Geometry check sheet. Reference: the model listing, model coordinates, mm. Coordinates: 2 decimals unless noted, no trailing zeros. Loops run counter-clockwise (first coordinate to the right, second up) from the corner with the lowest first, then second, coordinate; pieces in that order, holes last. Notation, with made-up numbers: (43, 40.5) - (52, 40.5) arc R14 cw to (52, 60.5) - close; hole circle Ø4 at (45, -37). An arc over 180 degrees is marked (long way). Write each question's results on one line, items separated by ' | '. Start each with the question number.
(1) Sectioned sample at C-C (y = 0). Enter the section's corners in (x, z), plus the area to 3 significant figures.
(2) Material ranges on probe 1 along Y at (x, z) = (19.6, -22); probe 2 along Y at (x, z) = (19.4, 26); probe 3 along Y at (x, z) = (19.35, 23), recorded low to high.
(3) Sectioned sample at B-B (x = 19.8). Enter the section's corners in (y, z), plus the area to 3 significant figures.
(4) Go/stop test with a flat-tipped pin: pin 1 Ø2.5 at (y, z) = (19, -28) entering from +X. Record where the tip stops, or that it passes through.
(5) Sectioned sample at A-A (z = 24). Enter the section's corners in (x, y).
from build123d import *

# Parameters (mm, degrees)
SKETCH_1_W                = 65
SKETCH_1_H                = 48
EXTRUDE_1_DEPTH           = 20
SKETCH_2_W                = 6
SKETCH_2_H                = 27.1
CUT_EXTRUDE_1_DEPTH       = 80
CUT_EXTRUDE_2_DEPTH       = 80
SKETCH_4_R                = 1.2
CUT_EXTRUDE_3_DEPTH       = 6
HOLE_WIZARD_1_D           = 3.4
HOLE_WIZARD_1_CBORE_D     = 6
HOLE_WIZARD_1_CBORE_DEPTH = 5
FILLET_1_R                = 5
SKETCH_9_W                = 19.082133463
SKETCH_9_H                = 84.157101427
CUT_EXTRUDE_6_DEPTH       = 120
SKETCH_10_W               = 25.015989719
SKETCH_10_H               = 30.267159573
EXTRUDE_2_DEPTH           = 1
SKETCH_11_R               = 1.6
CUT_EXTRUDE_7_DEPTH       = 120
FILLET_2_R                = 2


with BuildPart() as part:
    # 草图1 → 凸台-拉伸1 (new body)
    with BuildSketch(Plane(origin=(0, 0, 0), x_dir=(0, 0, -1), z_dir=(1, 0, 0))):
        Rectangle(SKETCH_1_W, SKETCH_1_H)
    extrude(amount=EXTRUDE_1_DEPTH)

    # 草图2 → 切除-拉伸1 (cut)
    with BuildSketch(Plane(origin=(0, 0, -32.5), x_dir=(-1, 0, 0), z_dir=(0, 0, -1))):
        Rectangle(SKETCH_2_W, SKETCH_2_H)
    extrude(amount=-CUT_EXTRUDE_1_DEPTH, mode=Mode.SUBTRACT)

    # 草图3 → 切除-拉伸2 (cut)
    with BuildSketch(Plane(origin=(20, 0, 0), x_dir=(0, 0, -1), z_dir=(1, 0, 0))):
        Polygon((-26.5, -9), (-21.5, -9), (-21.5, 9), (-26.5, 9), (-26.5, 5.5), (-32.5, 5.5), (-32.5, -5.5), (-26.5, -5.5), align=None)
    extrude(amount=-CUT_EXTRUDE_2_DEPTH, mode=Mode.SUBTRACT)

    # 草图4 → 切除-拉伸3 (cut)
    with BuildSketch(Plane(origin=(20, 0, 0), x_dir=(0, 0, -1), z_dir=(1, 0, 0))):
        with Locations((22, 0)):
            Circle(SKETCH_4_R)
    extrude(amount=-CUT_EXTRUDE_3_DEPTH, mode=Mode.SUBTRACT)

    # 打孔尺寸(%根据)开槽圆柱头螺钉的类型1 (through all)
    with Locations(Plane(origin=(20, 0, 0), x_dir=(0, 0, -1), z_dir=(1, 0, 0))):
        with Locations((7.35, -10), (-7.65, -10), (-7.65, 10), (7.35, 10)):
            CounterBoreHole(HOLE_WIZARD_1_D / 2, HOLE_WIZARD_1_CBORE_D / 2, HOLE_WIZARD_1_CBORE_DEPTH)

    # 圆角1
    fillet_1_edges = [part.edges().sort_by_distance(p)[0] for p in [
        (10, -24, -32.5),
        (10, 24, -32.5),
    ]]
    fillet(fillet_1_edges, radius=FILLET_1_R)

    # 草图9 → 切除-拉伸6 (cut)
    with BuildSketch(Plane(origin=(0, 24, 0), x_dir=(1, 0, 0), z_dir=(0, 1, 0))):
        with Locations((9.458933268, -0.081547579)):
            Rectangle(SKETCH_9_W, SKETCH_9_H)
    extrude(amount=-CUT_EXTRUDE_6_DEPTH, mode=Mode.SUBTRACT)

    # 草图10 → 凸台-拉伸2 (add)
    with BuildSketch(Plane.ZY.offset(-19)):
        with Locations((0.80226206, -0.656396231)):
            Rectangle(SKETCH_10_W, SKETCH_10_H)
    extrude(amount=-EXTRUDE_2_DEPTH)

    # 草图11 → 切除-拉伸7 (cut)
    with BuildSketch(Plane.ZY.offset(-19)):
        with Locations((-28, 19)):
            Circle(SKETCH_11_R)
        with Locations((-28, -19)):
            Circle(SKETCH_11_R)
        with Locations((27, -19)):
            Circle(SKETCH_11_R)
        with Locations(Location((27, 19, 0), (0, 0, 180))):
            Circle(SKETCH_11_R)
    extrude(amount=-CUT_EXTRUDE_7_DEPTH, mode=Mode.SUBTRACT)

    # 圆角2
    fillet_2_edges = [part.edges().sort_by_distance(p)[0] for p in [
        (19.5, -24, 32.5),
        (19.5, 24, 32.5),
    ]]
    fillet(fillet_2_edges, radius=FILLET_2_R)


solid = part.part
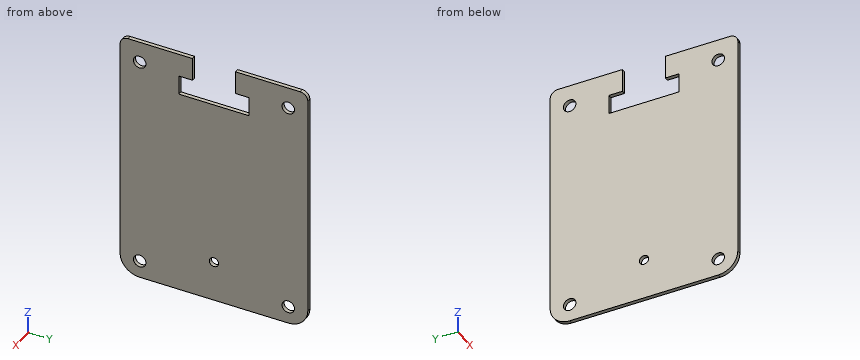
Outcome:
1) outline: (19, -32.5) - (20, -32.5) - (20, -23.2) - (19, -23.2) - close; (19, -20.8) - (20, -20.8) - (20, 21.5) - (19, 21.5) - close | area: 51.6 mm2
2) probe 1: y = -24 to -1.2, 1.2 to 24 | probe 2: y = -24 to -20.25, -17.75 to -9, 9 to 17.75, 20.25 to 24 | probe 3: y = -24 to -9, 9 to 24
3) outline: (-24, -27.5) arc R5 ccw to (-19, -32.5) - (19, -32.5) arc R5 ccw to (24, -27.5) - (24, 30.5) arc R2 ccw to (22, 32.5) - (5.5, 32.5) - (5.5, 26.5) - (9, 26.5) - (9, 21.5) - (-9, 21.5) - (-9, 26.5) - (-5.5, 26.5) - (-5.5, 32.5) - (-22, 32.5) arc R2 ccw to (-24, 30.5) - close; hole circle Ø3.2 at (-19, -28); hole circle Ø3.2 at (-19, 27); hole circle Ø2.4 at (0, -22); hole circle Ø3.2 at (19, -28); hole circle Ø3.2 at (19, 27) | area: 2,910 mm2
4) pin 1: passes through
5) outline: (19, -24) - (20, -24) - (20, -9) - (19, -9) - close; (19, 9) - (20, 9) - (20, 24) - (19, 24) - close
